For this review, use the dimensioned drawing (mm, ordinates from the lowest corner) and the shaded views. A direction names the side the tool comes from. Give positions to 0.01 mm unless a question says otherwise; leave off trailing zeros. Order: outer loops, then holes, each group sorted by start corner. A loop starts at its lowest first (then second) coordinate and runs counter-clockwise, first axis right, second up. Notation, with made-up numbers: (39, 16.25) -> (54, 16.25) arc R19 ccw to (54, 43.25) -> close; hole circle Ø4 at (20, 35). An arc over 180 degrees is marked (long way). One line per item, written item: value. Start each with the question number.
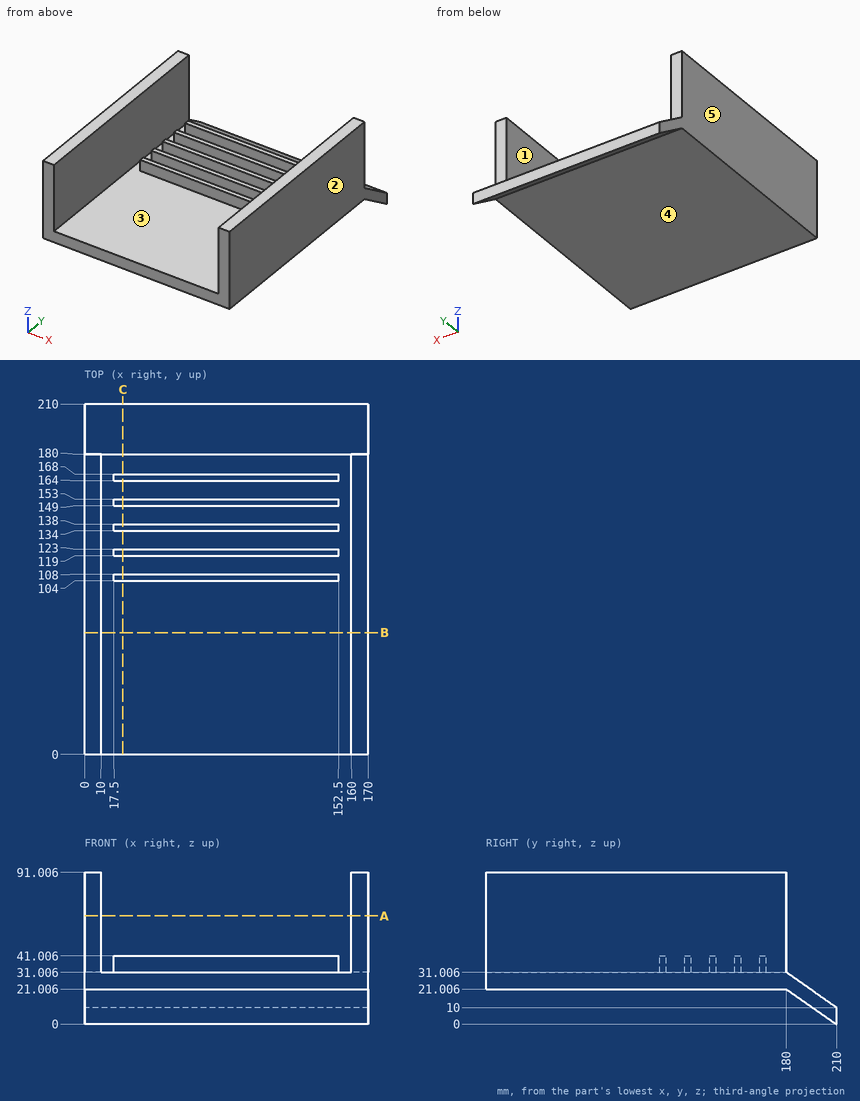
Q1. Take a section at B-B (y = 73). State the section outline as (x, z) points, and give its area (3 significant figures).
Q2. Take a section at C-C (x = 23). State the section outline as (y, z) points.
Q3. For line 1 along Y through (x, z) = (135, 40); line 2 along X through (y, z) = (54, 40); line 3 along Z through (x, y) = (11.5, 101.5), list the stretches that pass through material, from the lowest coordinate up.
Q4. Mouldability with a two-part tool opening along X and no side actions: class the marked faces 3, 4 and 5 as pulls with the +X half, pulls with the -X half, needs draft (parallel to the pull), parting line crosses it, or undercut.
Q5. For the marked faces 1 and 2, list the 3-axis set-ups (+Z, -Z, +X, -X, +Y, -Y) from which the entire face can be reached by the end or side of a thin tool; tool diameter is ignored.
Q6. For pin 1 Ø8 at (x, z) = (115.5, 36.5) entering from -Y; pin 2 Ø12 at (x, y) = (85, 48.5) entering from +Z; pin 3 Ø6 at (x, z) = (119, 10.5) entering from +Y; pin 4 Ø3 at (x, y) = (110, 121) entering from +Z, all flat-tipped, find the tip position at first contact; note any pin that passes through.
Q7. Take a section at A-A (z = 65). State the section outline as (x, y) points.
Answers below:
1. outline: (0, 21.01) -> (170, 21.01) -> (170, 91.01) -> (160, 91.01) -> (160, 31.01) -> (10, 31.01) -> (10, 91.01) -> (0, 91.01) -> close
1. area: 2,900 mm²
2. outline: (0, 21.01) -> (180, 21.01) -> (210, 0) -> (210, 10) -> (180, 31.01) -> (168, 31.01) -> (168, 41.01) -> (164, 41.01) -> (164, 31.01) -> (153, 31.01) -> (153, 41.01) -> (149, 41.01) -> (149, 31.01) -> (138, 31.01) -> (138, 41.01) -> (134, 41.01) -> (134, 31.01) -> (123, 31.01) -> (123, 41.01) -> (119, 41.01) -> (119, 31.01) -> (108, 31.01) -> (108, 41.01) -> (104, 41.01) -> (104, 31.01) -> (0, 31.01) -> close
3. line 1: y = 104 to 108, 119 to 123, 134 to 138, 149 to 153, 164 to 168
3. line 2: x = 0 to 10, 160 to 170
3. line 3: z = 21.01 to 31.01
4. face 3: undercut
4. face 4: needs draft
4. face 5: pulls with the -X half
5. face 1: +Z, +Y, -Y
5. face 2: +Z, -Z, +X, +Y, -Y
6. pin 1: stops at y = 104
6. pin 2: stops at z = 31.01
6. pin 3: stops at y = 210
6. pin 4: stops at z = 41.01
7. outline: (0, 0) -> (10, 0) -> (10, 180) -> (0, 180) -> close; (160, 0) -> (170, 0) -> (170, 180) -> (160, 180) -> close
